The model under review builds one solid part; all positions refer to its coordinate system, in mm. Face numbers are marked on the shaded views. A direction names the side the tool comes from. Coordinates: 2 decimals unless noted, no trailing zeros. Order: outer loops, then holes, each group sorted by start corner. A loop starts at its lowest first (then second) coordinate and runs counter-clockwise, first axis right, second up. Notation, with made-up numbers: (-26, 8.25) - (27, 8.25) arc R19 cw to (27, 13.25) - close; hole circle Ø8 at (76, 55.25). An arc over 180 degrees is marked (long way). Answer in a Markdown table with one row per item.
```python
from build123d import *

# Parameters (mm, degrees)
BLOCK_EXTRUDE_42_DEPTH     = 42
THROUGH_WINDOW_CUT_DEPTH   = 97.254870007
POCKET_20X7_SKETCH_W       = 20
POCKET_20X7_SKETCH_H       = 7
POCKET_20X7_DEPTH_10_DEPTH = 10
SIDE_SLOT_SKETCH_W         = 26
SIDE_SLOT_SKETCH_H         = 10
SIDE_SLOT_CUT_26X8_DEPTH   = 90.520947269


with BuildPart() as part:
    # Block Profile Sketch → Block Extrude 42 (new body)
    with BuildSketch(Plane.XY):
        with BuildLine():
            Line((0, 0), (16.875388203, 0))
            ThreePointArc((16.875388203, 0), (37, 9), (57.124611797, 0))
            Line((57.124611797, 0), (74, 0))
            Line((74, 0), (74, -10))
            Line((74, -10), (65, -10))
            Line((65, -10), (65, -26))
            Line((65, -26), (74, -26))
            Line((74, -26), (74, -36))
            Line((74, -36), (57.124611797, -36))
            ThreePointArc((57.124611797, -36), (37, -45), (16.875388203, -36))
            Line((16.875388203, -36), (0, -36))
            Line((0, -36), (0, -26))
            Line((0, -26), (9, -26))
            Line((9, -26), (9, -10))
            Line((9, -10), (0, -10))
            Line((0, -10), (0, 0))
        make_face()
    extrude(amount=-BLOCK_EXTRUDE_42_DEPTH)

    # Through Window Sketch → Through Window Cut (cut, through all)
    with BuildSketch(Plane.XY):
        Polygon((47, -10), (54, -10), (54, -26), (20, -26), (20, -10), (27, -10), align=None)
    extrude(amount=-THROUGH_WINDOW_CUT_DEPTH, mode=Mode.SUBTRACT)

    # Pocket 20x7 Sketch → Pocket 20x7 Depth 10 (cut)
    with BuildSketch(Plane.XY):
        with Locations((37, -6.5)):
            Rectangle(POCKET_20X7_SKETCH_W, POCKET_20X7_SKETCH_H)
    extrude(amount=-POCKET_20X7_DEPTH_10_DEPTH, mode=Mode.SUBTRACT)

    # Side Slot Sketch → Side Slot Cut 26x8 (cut, through all)
    with BuildSketch(Plane.ZY.offset(-9)):
        with Locations((-21, -18.075177639)):
            Rectangle(SIDE_SLOT_SKETCH_W, SIDE_SLOT_SKETCH_H)
    extrude(amount=-SIDE_SLOT_CUT_26X8_DEPTH, mode=Mode.SUBTRACT)


solid = part.part
```
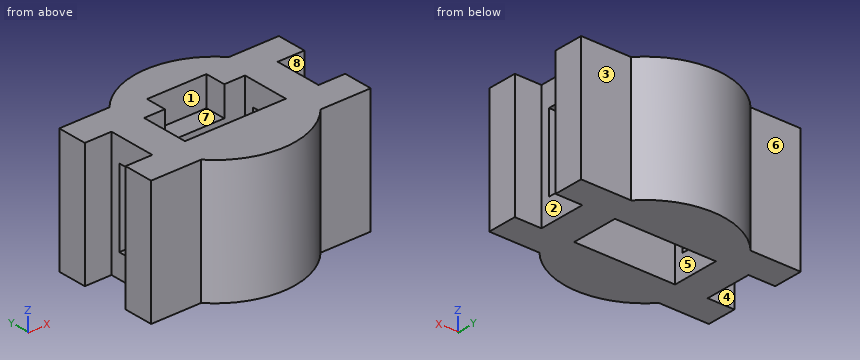
Item 1: Mouldability with a two-part tool opening along X and no side actions: class the marked faces 1, 2 and 3 as +X half, -X half, draft (parallel to the pull), parting line (faces both ways), or undercut.
Check values:
| item | result |
|---|---|
| face 1 | undercut |
| face 2 | +X half |
| face 3 | draft |
Item 2: Clearance check with flat-ended pins moving along their axes: pin 1 Ø2.5 at (x, z) = (4, -26) entering from -Y; pin 2 Ø5 at (x, z) = (61.5, -30.5) entering from +Y; pin 3 Ø1 at (y, z) = (-5.5, -6) entering from -X; pin 4 Ø12 at (x, z) = (59.5, -27) entering from +Y. State where each tip first meets the part, or that it passes through.
Check values:
| item | result |
|---|---|
| pin 1 | y = -36 |
| pin 2 | y = 0 |
| pin 3 | x = 0 |
| pin 4 | y = 3.37 |
Item 3: We need section A-A, the plane z = -18.5. Write out the cut boundary in (x, y).
Check values:
| item | result |
|---|---|
| outline | (0, -36) - (16.88, -36) arc R27 ccw to (57.12, -36) - (74, -36) - (74, -26) - (65, -26) - (65, -23.08) - (54, -23.08) - (54, -26) - (20, -26) - (20, -23.08) - (9, -23.08) - (9, -26) - (0, -26) - close; (0, -10) - (9, -10) - (9, -13.08) - (20, -13.08) - (20, -10) - (54, -10) - (54, -13.08) - (65, -13.08) - (65, -10) - (74, -10) - (74, 0) - (57.12, 0) arc R27 ccw to (16.88, 0) - (0, 0) - close |
Item 4: We need section D-D, the plane z = -35. Write out the cut boundary in (x, y).
Check values:
| item | result |
|---|---|
| outline | (0, -36) - (16.88, -36) arc R27 ccw to (57.12, -36) - (74, -36) - (74, -26) - (65, -26) - (65, -10) - (74, -10) - (74, 0) - (57.12, 0) arc R27 ccw to (16.88, 0) - (0, 0) - (0, -10) - (9, -10) - (9, -26) - (0, -26) - close; hole (20, -26) - (54, -26) - (54, -10) - (20, -10) - close |
Item 5: We need section B-B, the plane y = -14. Write out the cut boundary in (x, z).
Check values:
| item | result |
|---|---|
| outline | (9, -42) - (20, -42) - (20, -34) - (9, -34) - close; (9, -8) - (20, -8) - (20, 0) - (9, 0) - close; (54, -42) - (65, -42) - (65, -34) - (54, -34) - close; (54, -8) - (65, -8) - (65, 0) - (54, 0) - close |
Item 6: To check wall thickness, follow line 1 (Y direction, x = 68.5, z = -1.5); line 2 (Z direction, x = 55, y = -22); line 3 (X direction, y = -12, z = -7). State the ranges of each line that lie inside material, in increasing order. Write a range as from..to.
Check values:
| item | result |
|---|---|
| line 1 | -36..-26, -10..0 |
| line 2 | -42..-34, -8..0 |
| line 3 | 9..20, 54..65 |
Item 7: We need section C-C, the plane x = 68. Write out the cut boundary in (y, z).
Check values:
| item | result |
|---|---|
| outline | (-36, -42) - (-26, -42) - (-26, 0) - (-36, 0) - close; (-10, -42) - (0, -42) - (0, 0) - (-10, 0) - close |
Item 8: Tool access review of the marked faces 4, 5, 6, 7 and 8: name each direction out of +Z, -Z, +X, -X, +Y, -Y from which nothing blocks a thin tool from reaching the whole face with its end or side.
Check values:
| item | result |
|---|---|
| face 4 | +Z, -Z, -X |
| face 5 | +Z, -Z |
| face 6 | +Z, -Z, -X, +Y |
| face 7 | +Z |
| face 8 | +Z, -Z, +X |
